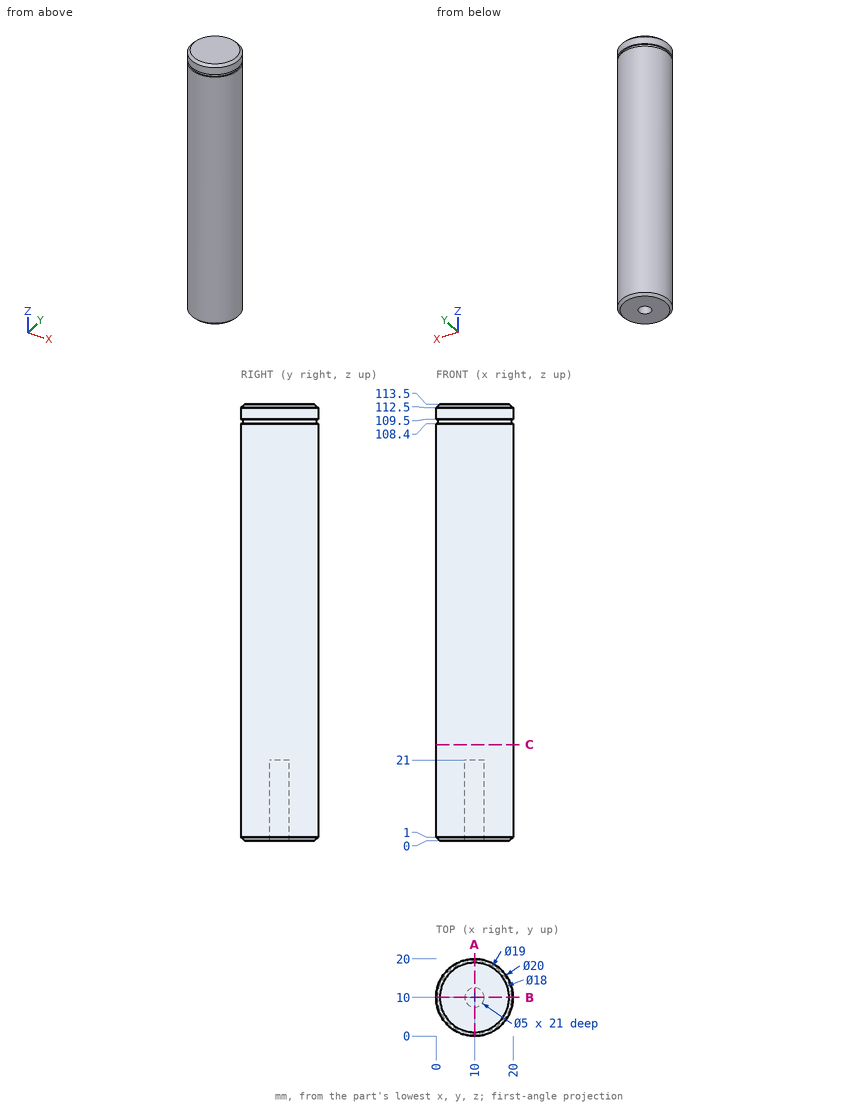
Geometry check sheet. Reference: drawing and pictorial views, mm from the part's lowest x, y, z. Give positions to 0.01 mm unless a question says otherwise; leave off trailing zeros. Loops run counter-clockwise (first coordinate to the right, second up) from the corner with the lowest first, then second, coordinate; pieces in that order, holes last. Notation, with made-up numbers: M 1,72 L 35,72 A24 ccw 35,83 Z; hole C 27.5,59.25 d10. An arc over 180 degrees is marked long. One line per question, with ' | ' between items.
Item 1: Section check C-C, the plane z = 25. Record the cut outline in (x, y).
Completed:
outline: C 10,10 d20
Item 2: Thickness scan on line 1 (Y direction, x = 10, z = 5.75); line 2 (Z direction, x = 10.5, y = 11.5); line 3 (Z direction, x = 2, y = 15.75). Record the ranges inside material, lowest first. Write a range as [from, to].
Completed:
line 1: y = [0, 7.5], [12.5, 20] | line 2: z = [21, 113.5] | line 3: z = [0.85, 108.4], [109.5, 112.65]
Item 3: Depth check by flat-ended pin: P1, Ø2.5, axis at x = 9, y = 9.5, coming from the -Z side; P2, Ø12, axis at y = 17.5, z = 49, coming from the -X side; P3, Ø1.5, axis at x = 6.5, z = 47.5, coming from the +Y side. Enter the tip coordinate at first touch or a pass-through.
Completed:
P1: stops at z = 21 | P2: stops at x = 0.11 | P3: stops at y = 19.61
Item 4: Section check A-A, the plane x = 10. Record the cut outline in (y, z), plus the area to 3 significant figures.
Completed:
outline: M 0,1 L 1,0 L 7.5,0 L 7.5,21 L 12.5,21 L 12.5,0 L 19,0 L 20,1 L 20,108.4 L 19.5,108.4 L 19.5,109.5 L 20,109.5 L 20,112.5 L 19,113.5 L 1,113.5 L 0,112.5 L 0,109.5 L 0.5,109.5 L 0.5,108.4 L 0,108.4 Z | area: 2,160 mm^2
